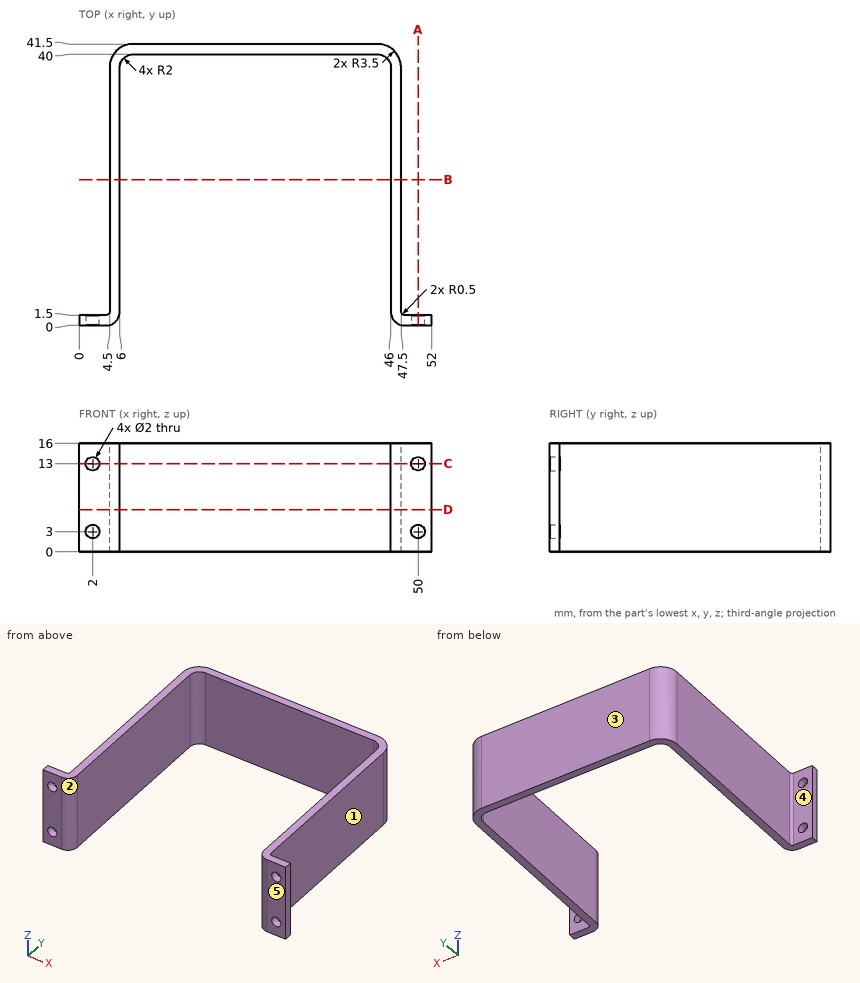
Print and shaded views of the part. All mm, measured from the part's lowest x, y and z. A direction names the side the tool comes from. Coordinates: 2 decimals unless noted, no trailing zeros. Loops run counter-clockwise (first coordinate to the right, second up) from the corner with the lowest first, then second, coordinate; pieces in that order, holes last. Notation, with made-up numbers: (22, 5.25) -> (65, 5.25) arc R14 ccw to (65, 16.25) -> close; hole circle Ø11 at (62.25, 35.5). An arc over 180 degrees is marked (long way). Use one line per item in the form item = value. Start each with the question number.
(1) Cut at A-A on x = 50. Give the cut face in (y, z), and give its area (3 significant figures).
(2) Cut at B-B on y = 21.5. Give the cut face in (x, z).
(3) Cut at C-C on z = 13. Give the cut face in (x, y), and give its area (3 significant figures).
(4) Cut at D-D on z = 6.25. Give the cut face in (x, y).
(5) Flat gauge pins, fed straight in: pin 1 (5 mm diameter, centred on y = 13.5, z = 4, fed in from -X); pin 2 (6 mm diameter, centred on x = 16.5, z = 13.5, fed in from -Y); pin 3 (1.2 mm diameter, centred on x = 50.5, z = 7, fed in from +Y). Where does each tip first touch, or does it go through?
(6) Probe probe 1 along Z at (x, y) = (2, 0.95); probe 2 along X at (y, z) = (32.5, 4); probe 3 along Y at (x, z) = (21, 5). List the from-to ranges inside material, lowest first. Write a range as from..to.
(7) Tool access for the marked faces 1, 2, 3, 4 and 5: list every direction of +Z, -Z, +X, -X, +Y, -Y with a clear straight run to the whole face (end or side of a thin tool).
Values:
q1.outline = (0, 0) -> (1.5, 0) -> (1.5, 2) -> (0, 2) -> close; (0, 4) -> (1.5, 4) -> (1.5, 12) -> (0, 12) -> close; (0, 14) -> (1.5, 14) -> (1.5, 16) -> (0, 16) -> close
q1.area = 18.0 mm2
q2.outline = (4.5, 0) -> (6, 0) -> (6, 16) -> (4.5, 16) -> close; (46, 0) -> (47.5, 0) -> (47.5, 16) -> (46, 16) -> close
q3.outline = (0, 0) -> (1, 0) -> (1, 1.5) -> (0, 1.5) -> close; (3, 0) -> (4, 0) arc R2 ccw to (6, 2) -> (6, 38) arc R2 cw to (8, 40) -> (44, 40) arc R2 cw to (46, 38) -> (46, 2) arc R2 ccw to (48, 0) -> (49, 0) -> (49, 1.5) -> (48, 1.5) arc R0.5 cw to (47.5, 2) -> (47.5, 38) arc R3.5 ccw to (44, 41.5) -> (8, 41.5) arc R3.5 ccw to (4.5, 38) -> (4.5, 2) arc R0.5 cw to (4, 1.5) -> (3, 1.5) -> close; (51, 0) -> (52, 0) -> (52, 1.5) -> (51, 1.5) -> close
q3.area = 187 mm2
q4.outline = (0, 0) -> (4, 0) arc R2 ccw to (6, 2) -> (6, 38) arc R2 cw to (8, 40) -> (44, 40) arc R2 cw to (46, 38) -> (46, 2) arc R2 ccw to (48, 0) -> (52, 0) -> (52, 1.5) -> (48, 1.5) arc R0.5 cw to (47.5, 2) -> (47.5, 38) arc R3.5 ccw to (44, 41.5) -> (8, 41.5) arc R3.5 ccw to (4.5, 38) -> (4.5, 2) arc R0.5 cw to (4, 1.5) -> (0, 1.5) -> close
q5.pin_1 = 4.5
q5.pin_2 = 40
q5.pin_3 = 1.5
q6.probe_1 = 0..2, 4..12, 14..16
q6.probe_2 = 4.5..6, 46..47.5
q6.probe_3 = 40..41.5
q7.face_1 = +Z, -Z, +X, +Y
q7.face_2 = +Z, -Z, -Y
q7.face_3 = +Z, -Z, +X, -X, +Y
q7.face_4 = +Z, -Z, -X, +Y
q7.face_5 = +Z, -Z, +X, -X, -Y
